from build123d import *

# Parameters (mm, degrees)
SKETCH_1_R      = 5
EXTRUDE_1_DEPTH = 5


with BuildPart() as part:
    # 草图1 → 凸台-拉伸1 (new body)
    with BuildSketch(Plane.XY):
        with BuildLine():
            Line((0, 0), (30, 0))
            Line((30, 0), (30, 55))
            ThreePointArc((30, 55), (15, 70), (0, 55))
            Line((0, 55), (0, 0))
        make_face()
        with Locations((15, 55)):
            Circle(SKETCH_1_R, mode=Mode.SUBTRACT)
    extrude(amount=EXTRUDE_1_DEPTH)


solid = part.part
Design review of the part built by this model. Coordinates are the model's own, in mm. Round coordinates to 2 decimals unless told otherwise and drop trailing zeros. Write each loop counter-clockwise with the first axis right and the second up, starting at its lowest first coordinate (ties: lowest second). Pieces come first, ordered by that corner, then holes. Notation, with made-up numbers: (48.25, 62.25) - (84.25, 62.25) arc R5 cw to (84.25, 66.25) - close; hole circle Ø2 at (25.25, 34). An arc over 180 degrees is marked (long way). Return JSON: item names as keys, results as strings. Group by question number.
Item 1: We need section C-C on y = 64. Write out the cut boundary in (x, z).
Item 2: The part is to be moulded in two halves that separate along X. For faces 1 (the face through (18, 59, 2)), 2 (the face through (30, 27, 2)), 3 (the face through (15, 35, 0)), say which applies: pulls with the +X half, pulls with the -X half, needs draft (parallel to the pull), parting line crosses it, or undercut.
Item 3: We need section A-A on x = 15. Write out the cut boundary in (y, z).
Item 4: We need section B-B on z = 1.4. Write out the cut boundary in (x, y), and give its area (3 significant figures).
Item 5: We need section D-D on x = 21.5. Write out the cut boundary in (y, z).
Item 6: Insertion check: P1, Ø3, axis at x = 9.5, z = 4, coming from the +Y side; P2, Ø3, axis at x = 3.5, z = 1.5, coming from the +Y side; P3, Ø2, axis at x = 5.5, z = 1, coming from the +Y side. Each pin has a flat end and moves straight along its axis. Give the tip position at first contact, or say it passes through.
Item 7: For probe 1 along Y at (x, z) = (15, 3.2); probe 2 along X at (y, z) = (54.5, 2.3); probe 3 along Y at (x, z) = (11.25, 2.25), list the stretches that pass through material, from the lowest coordinate up. Write a range as [from, to].
Model answer:
{
 "1": {"outline": "(3, 0) - (27, 0) - (27, 5) - (3, 5) - close"},
 "2": {"face 1": "undercut", "face 2": "pulls with the +X half", "face 3": "needs draft"},
 "3": {"outline": "(0, 0) - (50, 0) - (50, 5) - (0, 5) - close; (60, 0) - (70, 0) - (70, 5) - (60, 5) - close"},
 "4": {"outline": "(0, 0) - (30, 0) - (30, 55) arc R15 ccw to (0, 55) - close; hole circle Ø10 at (15, 55)", "area": "1,920 mm²"},
 "5": {"outline": "(0, 0) - (68.52, 0) - (68.52, 5) - (0, 5) - close"},
 "6": {"P1": "stops at y = 69.46", "P2": "stops at y = 66.18", "P3": "stops at y = 67.36"},
 "7": {"probe 1": "y = [0, 50], [60, 70]", "probe 2": "x = [0, 10.03], [19.97, 30]", "probe 3": "y = [0, 51.69], [58.31, 69.52]"}
}
